from build123d import *

# Parameters (mm, degrees)
EXTRUDE_1_DEPTH     = 10
SKETCH_2_R          = 6
CUT_EXTRUDE_1_DEPTH = 197.277864264
SKETCH_3_W          = 130
SKETCH_3_H          = 120
SKETCH_3_W_2        = 120
SKETCH_3_H_2        = 110
EXTRUDE_4_DEPTH     = 135
SKETCH_4_R          = 40
EXTRUDE_5_DEPTH     = 15
SKETCH_6_R          = 34
CUT_EXTRUDE_2_DEPTH = 20
SKETCH_7_R          = 40
EXTRUDE_6_DEPTH     = 15
SKETCH_8_R          = 34
CUT_EXTRUDE_3_DEPTH = 20
EXTRUDE_START       = 15
SKETCH_9_R          = 40
EXTRUDE_7_DEPTH     = 15
CUT_EXTRUDE_START   = -20
SKETCH_10_R         = 34
CUT_EXTRUDE_4_DEPTH = 20


with BuildPart() as part:
    # 草图1 → 凸台-拉伸1 (new body)
    with BuildSketch(Plane(origin=(0, 0, 0), x_dir=(1, 0, 0), z_dir=(0, 1, 0))):
        with BuildLine():
            Line((0, 120), (-12.5, 120))
            ThreePointArc((-12.5, 120), (-21.338834765, 116.338834765), (-25, 107.5))
            Line((-25, 107.5), (-25, 12.5))
            ThreePointArc((-25, 12.5), (-21.338834765, 3.661165235), (-12.5, 0))
            Line((-12.5, 0), (0, 0))
            Line((0, 0), (130, 0))
            Line((130, 0), (142.5, 0))
            ThreePointArc((142.5, 0), (151.338834765, 3.661165235), (155, 12.5))
            Line((155, 12.5), (155, 107.5))
            ThreePointArc((155, 107.5), (151.338834765, 116.338834765), (142.5, 120))
            Line((142.5, 120), (130, 120))
            Line((130, 120), (0, 120))
        make_face()
    extrude(amount=EXTRUDE_1_DEPTH)

    # 草图2 → 切除-拉伸1 (cut, through all)
    with BuildSketch(Plane(origin=(0, 10, 0), x_dir=(1, 0, 0), z_dir=(0, 1, 0))):
        with Locations(Location((-12.5, 107.5, 0), (0, 0, 270))):
            Circle(SKETCH_2_R)
        with Locations(Location((142.5, 107.5, 0), (0, 0, 270))):
            Circle(SKETCH_2_R)
        with Locations(Location((142.5, 12.5, 0), (0, 0, 270))):
            Circle(SKETCH_2_R)
        with Locations(Location((-12.5, 12.5, 0), (0, 0, 270))):
            Circle(SKETCH_2_R)
    extrude(amount=-CUT_EXTRUDE_1_DEPTH, mode=Mode.SUBTRACT)

    # 草图3 → 凸台-拉伸4 (add)
    with BuildSketch(Plane(origin=(0, 10, 0), x_dir=(1, 0, 0), z_dir=(0, 1, 0))):
        with Locations((65, 60)):
            Rectangle(SKETCH_3_W, SKETCH_3_H)
        with Locations((65, 60)):
            Rectangle(SKETCH_3_W_2, SKETCH_3_H_2, mode=Mode.SUBTRACT)
    extrude(amount=EXTRUDE_4_DEPTH)

    # 草图4 → 凸台-拉伸5 (add)
    with BuildSketch(Plane.XY):
        with Locations(Location((60, 95, 0), (0, 0, 180))):
            Circle(SKETCH_4_R)
    extrude(amount=EXTRUDE_5_DEPTH)

    # 草图6 → 切除-拉伸2 (cut)
    with BuildSketch(Plane.XY.offset(15)):
        with Locations((60, 95)):
            Circle(SKETCH_6_R)
    extrude(amount=-CUT_EXTRUDE_2_DEPTH, mode=Mode.SUBTRACT)

    # 草图7 → 凸台-拉伸6 (add)
    with BuildSketch(Plane(origin=(130, 0, 0), x_dir=(0, 0, -1), z_dir=(1, 0, 0))):
        with Locations(Location((50, 95, 0), (0, 0, 180))):
            Circle(SKETCH_7_R)
    extrude(amount=EXTRUDE_6_DEPTH)

    # 草图8 → 切除-拉伸3 (cut)
    with BuildSketch(Plane(origin=(145, 0, 0), x_dir=(0, 0, -1), z_dir=(1, 0, 0))):
        with Locations((50, 95)):
            Circle(SKETCH_8_R)
    extrude(amount=-CUT_EXTRUDE_3_DEPTH, mode=Mode.SUBTRACT)

    # 草图9 → 凸台-拉伸7 (add)
    with BuildSketch(Plane(origin=(0, 0, -120), x_dir=(-1, 0, 0), z_dir=(0, 0, -1)).offset(EXTRUDE_START)):
        with Locations((-60, 95)):
            Circle(SKETCH_9_R)
    extrude(amount=-EXTRUDE_7_DEPTH)

    # 草图10 → 切除-拉伸4 (cut)
    with BuildSketch(Plane(origin=(0, 0, -135), x_dir=(-1, 0, 0), z_dir=(0, 0, -1)).offset(CUT_EXTRUDE_START)):
        with Locations(Location((-60, 95, 0), (0, 0, 180))):
            Circle(SKETCH_10_R)
    extrude(amount=CUT_EXTRUDE_4_DEPTH, mode=Mode.SUBTRACT)


solid = part.part
Geometry check sheet. Reference: the model listing, model coordinates, mm. A direction names the side the tool comes from. Give positions to 0.01 mm unless a question says otherwise; leave off trailing zeros. Order: outer loops, then holes, each group sorted by start corner. A loop starts at its lowest first (then second) coordinate and runs counter-clockwise, first axis right, second up. Notation, with made-up numbers: (78.25, 0) - (134.25, 0) arc R11 cw to (134.25, 9) - close; hole circle Ø1 at (29, 50). An arc over 180 degrees is marked (long way). Use one line per item in the form item = value.
1) Draft check along X on faces 1 (the face through (151.241, 4.93, -3.565)), 2 (the face through (-21.435, 4.93, -3.759)), 3 (the face through (33.02, 115.69, -124.86)). Enter one of: released by +X, released by -X, zero draft, split by the parting line, or undercut.
Working result:
face_1 = released by +X
face_2 = released by -X
face_3 = undercut
2) Sectioned sample at A-A (y = 95). Count the separate pieces of the cut face and the enclosed holes in it, and give its area (3 significant figures).
Working result:
separate_pieces = 3
enclosed_holes = 0
area = 1,920 mm^2
3) Sectioned sample at C-C (z = -50). Record the boundary of the cut face in (x, y), and give its area (3 significant figures).
Working result:
outline = (-25, 0) - (155, 0) - (155, 10) - (130, 10) - (130, 55) - (145, 55) - (145, 61) - (125, 61) - (125, 10) - (5, 10) - (5, 145) - (0, 145) - (0, 10) - (-25, 10) - close; (125, 129) - (145, 129) - (145, 135) - (130, 135) - (130, 145) - (125, 145) - close
area = 2,990 mm^2
4) Material ranges on probe 1 along Z at (x, y) = (142, 4); probe 2 along Z at (x, y) = (36, 11); probe 3 along X at (y, z) = (5.25, -12.5), recorded low to high. Write a range as from..to.
Working result:
probe_1 = -120..-113.48, -101.52..-18.48, -6.52..0
probe_2 = -120..-115, -5..0
probe_3 = -25..-18.5, -6.5..136.5, 148.5..155
5) Sectioned sample at B-B (x = 60). Record the boundary of the cut face in (y, z), and give its area (3 significant figures).
Working result:
outline = (0, -120) - (55, -120) - (55, -135) - (61, -135) - (61, -115) - (10, -115) - (10, -5) - (61, -5) - (61, 15) - (55, 15) - (55, 0) - (0, 0) - close; (129, -135) - (135, -135) - (135, -120) - (145, -120) - (145, -115) - (129, -115) - close; (129, -5) - (145, -5) - (145, 0) - (135, 0) - (135, 15) - (129, 15) - close
area = 2,230 mm^2
6) Depth check by flat-ended pin: pin 1 Ø12.5 at (x, z) = (138.5, -87) entering from +Y; pin 2 Ø1 at (y, z) = (31, -21.5) entering from -X; pin 3 Ø10 at (x, z) = (110.5, -60) entering from +Y. Enter the tip coordinate at first touch or a pass-through.
Working result:
pin_1 = 120.58
pin_2 = 0
pin_3 = 10
7) Access from +Z, -Z, +X, -X, +Y, -Y to the whole of each face (thin tool, end or side, straight path). Record for faces 4 (the face through (21.847, 107.015, -127.605)), 5 (the face through (21.847, 82.985, 7.395)), 6 (the face through (64, 10, -61)).
Working result:
face_4 = -Z
face_5 = +Z
face_6 = +Y
